from build123d import *

# Parameters (mm, degrees)
SKETCH1_R           = 6.5
BOSS_EXTRUDE1_DEPTH = 2.5


with BuildPart() as part:
    # Sketch1 → Boss-Extrude1 (new, symmetric)
    with BuildSketch(Plane.XY):
        with BuildLine():
            Line((167.313008395, 349.517677982), (183.912598704, 421.418402931))
            ThreePointArc((183.912598704, 421.418402931), (207.899021087, 436.40678314), (222.887401296, 412.420360758))
            Line((222.887401296, 412.420360758), (203.766561676, 329.598905251))
            ThreePointArc((203.766561676, 329.598905251), (185.806892251, 340.047127311), (167.313008395, 349.517677982))
        make_face()
        with Locations((203.4, 416.919381844)):
            Circle(SKETCH1_R, mode=Mode.SUBTRACT)
    extrude(amount=BOSS_EXTRUDE1_DEPTH, both=True)


solid = part.part
For this review, take the finished solid that the model builds, in its own axes (mm). Give positions to 0.01 mm unless a question says otherwise; leave off trailing zeros. Loops run counter-clockwise (first coordinate to the right, second up) from the corner with the lowest first, then second, coordinate; pieces in that order, holes last. Notation, with made-up numbers: (-25.5, 60) -> (-1.5, 60) arc R24 ccw to (-1.5, 89) -> close; hole circle Ø8 at (47.5, 7.25). An arc over 180 degrees is marked (long way). One line per question, with ' | ' between items.
1) We need section C-C (x = 199). Write out the cut boundary in (y, z), plus the area to 3 significant figures.
Resolved:
outline: (332.5, -2.5) -> (412.14, -2.5) -> (412.14, 2.5) -> (332.5, 2.5) -> close; (421.7, -2.5) -> (436.43, -2.5) -> (436.43, 2.5) -> (421.7, 2.5) -> close | area: 472 mm2
2) We need section D-D (y = 429.5). Write out the cut boundary in (x, z), plus the area to 3 significant figures.
Resolved:
outline: (187.85, -2.5) -> (218.95, -2.5) -> (218.95, 2.5) -> (187.85, 2.5) -> close | area: 155 mm2
3) We need section A-A (x = 208). Write out the cut boundary in (y, z).
Resolved:
outline: (347.94, -2.5) -> (412.33, -2.5) -> (412.33, 2.5) -> (347.94, 2.5) -> close; (421.51, -2.5) -> (436.38, -2.5) -> (436.38, 2.5) -> (421.51, 2.5) -> close
4) The part is to be moulded in two halves that separate along X. For faces 1 (the flat face through (196, 384, -2.5)), 2 (the cylindrical face through (206.894, 422.4, -0.035)), 3 (the flat face through (213.46, 371.59, 0.04)), say which applies: +X half, -X half, draft (parallel to the pull), parting line (faces both ways), or undercut.
Resolved:
face 1: draft | face 2: undercut | face 3: +X half
5) Insertion check: pin 1 Ø1.5 at (y, z) = (341, 2) entering from +X. The pin has a flat end and moves straight along its axis. Give the tip position at first contact, or say it passes through.
Resolved:
pin 1: stops at x = 206.57
6) To check wall thickness, follow probe 1 along Y at (x, z) = (203.4, 0.75); probe 2 along X at (y, z) = (358, 0.85); probe 3 along X at (y, z) = (403, -2.3). State the ranges of each line that lie inside material, in increasing order.
Resolved:
probe 1: y = 329.83 to 410.42, 423.42 to 436.92 | probe 2: x = 169.27 to 210.32 | probe 3: x = 179.66 to 220.71
7) We need section B-B (z = -1.1). Write out the cut boundary in (x, y), plus the area to 3 significant figures.
Resolved:
outline: (167.31, 349.52) arc R387.5 cw to (203.77, 329.6) -> (222.89, 412.42) arc R20 ccw to (183.91, 421.42) -> close; hole circle Ø13 at (203.4, 416.92) | area: 3,660 mm2
